Work out the finished part from the listing and answer in its coordinate system (mm). Face numbers are marked on the shaded views. A direction names the side the tool comes from. Give positions to 0.01 mm unless a question says otherwise; leave off trailing zeros. Loops run counter-clockwise (first coordinate to the right, second up) from the corner with the lowest first, then second, coordinate; pieces in that order, holes last. Notation, with made-up numbers: M 31.25,17 L 51.25,17 A11 cw 51.25,34 Z; hole C 26.5,20 d10. An arc over 180 degrees is marked long. Answer in a Markdown table with one row per item. Add a question column.
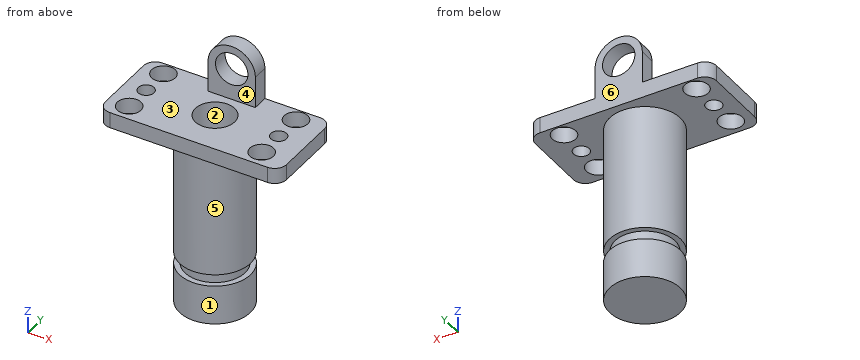
from build123d import *

# Parameters (mm, degrees)
FLANGE_PLATE_DEPTH      = 10
SHAFT_45_SKETCH_R       = 22.5
SHAFT_45_DEPTH          = 80
GROOVE_NECK_SKETCH_R    = 19.038570364
GROOVE_NECK_38_DEPTH    = 7.5
SHAFT_END_SKETCH_R      = 22.5
SHAFT_END_45_DEPTH      = 25
CENTRE_BORE_SKETCH_R    = 12.5
CENTRE_BORE_25_DEPTH    = 25
FLANGE_HOLES_SKETCH_R   = 7.5
FLANGE_HOLES_SKETCH_R_2 = 5
FLANGE_HOLES_6X_DEPTH   = 25
LUG_DEPTH               = 10
LUG_HOLE_SKETCH_R       = 10.286699657
LUG_HOLE_20_6_DEPTH     = 10


with BuildPart() as part:
    # Flange Plate Sketch → Flange Plate (new body)
    with BuildSketch(Plane.XY):
        with BuildLine():
            Line((0, 0), (50, 0))
            ThreePointArc((50, 0), (55.303300859, 2.196699141), (57.5, 7.5))
            Line((57.5, 7.5), (57.5, 47.5))
            ThreePointArc((57.5, 47.5), (55.303300859, 52.803300859), (50, 55))
            Line((50, 55), (-50, 55))
            ThreePointArc((-50, 55), (-55.303300859, 52.803300859), (-57.5, 47.5))
            Line((-57.5, 47.5), (-57.5, 7.5))
            ThreePointArc((-57.5, 7.5), (-55.303300859, 2.196699141), (-50, 0))
            Line((-50, 0), (0, 0))
        make_face()
    extrude(amount=FLANGE_PLATE_DEPTH)

    # Shaft Ø45 Sketch → Shaft Ø45 (add)
    with BuildSketch(Plane(origin=(0, 0, 0), x_dir=(-1, 0, 0), z_dir=(0, 0, -1))):
        with Locations((0, 27.5)):
            Circle(SHAFT_45_SKETCH_R)
    extrude(amount=SHAFT_45_DEPTH)

    # Groove Neck Sketch → Groove Neck Ø38 (add)
    with BuildSketch(Plane(origin=(0, 0, -80), x_dir=(-1, 0, 0), z_dir=(0, 0, -1))):
        with Locations((0, 27.5)):
            Circle(GROOVE_NECK_SKETCH_R)
    extrude(amount=GROOVE_NECK_38_DEPTH)

    # Shaft End Sketch → Shaft End Ø45 (add)
    with BuildSketch(Plane(origin=(0, 0, -87.5), x_dir=(-1, 0, 0), z_dir=(0, 0, -1))):
        with Locations((0, 27.5)):
            Circle(SHAFT_END_SKETCH_R)
    extrude(amount=SHAFT_END_45_DEPTH)

    # Centre Bore Sketch → Centre Bore Ø25 (cut)
    with BuildSketch(Plane.XY.offset(10)):
        with Locations((0, 27.5)):
            Circle(CENTRE_BORE_SKETCH_R)
    extrude(amount=-CENTRE_BORE_25_DEPTH, mode=Mode.SUBTRACT)

    # Flange Holes Sketch → Flange Holes 6x (cut)
    with BuildSketch(Plane.XY.offset(10)):
        with Locations((39.858984169, 46.529450506)):
            Circle(FLANGE_HOLES_SKETCH_R)
        with Locations((39.858984169, 28.400041578)):
            Circle(FLANGE_HOLES_SKETCH_R_2)
        with Locations((39.858984169, 10.656364754)):
            Circle(FLANGE_HOLES_SKETCH_R)
        with Locations((-44.230614691, 10.656364754)):
            Circle(FLANGE_HOLES_SKETCH_R)
        with Locations((-44.230614691, 28.400041578)):
            Circle(FLANGE_HOLES_SKETCH_R_2)
        with Locations((-44.230614691, 46.529450506)):
            Circle(FLANGE_HOLES_SKETCH_R)
    extrude(amount=-FLANGE_HOLES_6X_DEPTH, mode=Mode.SUBTRACT)

    # Lug Sketch → Lug (add)
    with BuildSketch(Plane(origin=(0, 55, 0), x_dir=(1, 0, 0), z_dir=(0, 1, 0))):
        with BuildLine():
            Line((0, -10), (-15, -10))
            Line((-15, -10), (-15, -30))
            ThreePointArc((-15, -30), (0, -45), (15, -30))
            Line((15, -30), (15, -10))
            Line((15, -10), (0, -10))
        make_face()
    extrude(amount=-LUG_DEPTH)

    # Lug Hole Sketch → Lug Hole Ø20.6 (cut)
    with BuildSketch(Plane.XZ.offset(-45)):
        with Locations(Location((0, 30, 0), (0, 0, 270))):
            Circle(LUG_HOLE_SKETCH_R)
    extrude(amount=-LUG_HOLE_20_6_DEPTH, mode=Mode.SUBTRACT)


solid = part.part
(1) Which of the six approach directions +Z, -Z, +X, -X, +Y, -Y give full straight-line access (tool end or side, diameter ignored) to the marked faces 4, 5 and 6?
(2) Section C-C, the plane x = 37 is taken. Determine the outline of the cut face in (y, z), and give its area (3 significant figures).
(3) Section A-A, the plane x = 0 is taken. Determine the outline of the cut face in (y, z).
(4) Consider line 1 along Z through (x, y) = (28, 46); line 2 along Z through (x, y) = (3.5, 49.5); line 3 along X through (y, z) = (49, 30). Determine where each line is inside the solid, lowest interval first. Write a range as from..to.
(5) Section B-B, the plane y = 42.5 is taken. Determine the outline of the cut face in (x, z).
(6) Section D-D, the plane z = -24.5 is taken. Determine the outline of the cut face in (x, y).
(7) Each of these flat-tipped pins is pushed along its axis until it touches: P1, Ø24, axis at x = 4.5, z = 29, coming from the -Y side; P2, Ø4, axis at y = 14.5, z = -68, coming from the +X side; P3, Ø19.5, axis at x = -44.23, y = 10.66, coming from the +Z side; P4, Ø12, axis at x = -33.5, z = -27, coming from the +Y side. Where does it stop, or does it pass through?
(8) The mould has two halves that part along X. Classify the marked faces 1, 2 and 3: pulls with the +X half, pulls with the -X half, needs draft (parallel to the pull), parting line crosses it, or undercut.
Numbers:
| question | item | result |
|---|---|---|
| 1 | face 4 | +Z, +X, -X, -Y |
| 1 | face 5 | -Z |
| 1 | face 6 | +Z, -Z, +X, -X, +Y |
| 2 | outline | M 0,0 L 3.72,0 L 3.72,10 L 0,10 Z; M 17.59,0 L 24.3,0 L 24.3,10 L 17.59,10 Z; M 32.5,0 L 39.6,0 L 39.6,10 L 32.5,10 Z; M 53.46,0 L 55,0 L 55,10 L 53.46,10 Z |
| 2 | area | 191 mm² |
| 3 | outline | M 0,0 L 5,0 L 5,-80 L 8.46,-80 L 8.46,-87.5 L 5,-87.5 L 5,-112.5 L 50,-112.5 L 50,-87.5 L 46.54,-87.5 L 46.54,-80 L 50,-80 L 50,0 L 55,0 L 55,19.71 L 45,19.71 L 45,10 L 40,10 L 40,-15 L 15,-15 L 15,10 L 0,10 Z; M 45,40.29 L 55,40.29 L 55,45 L 45,45 Z |
| 4 | line 1 | z = 0..10 |
| 4 | line 2 | z = -112.5..-87.5, -80..20.33, 39.67..44.59 |
| 4 | line 3 | x = -15..-10.29, 10.29..15 |
| 5 | outline | M -57.5,0 L -50.56,0 L -50.56,10 L -57.5,10 Z; M -37.9,0 L -16.77,0 L -16.77,-80 L -11.72,-80 L -11.72,-87.5 L -16.77,-87.5 L -16.77,-112.5 L 16.77,-112.5 L 16.77,-87.5 L 11.72,-87.5 L 11.72,-80 L 16.77,-80 L 16.77,0 L 33.53,0 L 33.53,10 L -37.9,10 Z; M 46.18,0 L 57.5,0 L 57.5,10 L 46.18,10 Z |
| 6 | outline | C 0,27.5 d45 |
| 7 | P1 | stops at y = 45 |
| 7 | P2 | stops at x = 19.63 |
| 7 | P3 | stops at z = 10 |
| 7 | P4 | passes through |
| 8 | face 1 | parting line crosses it |
| 8 | face 2 | undercut |
| 8 | face 3 | needs draft |
